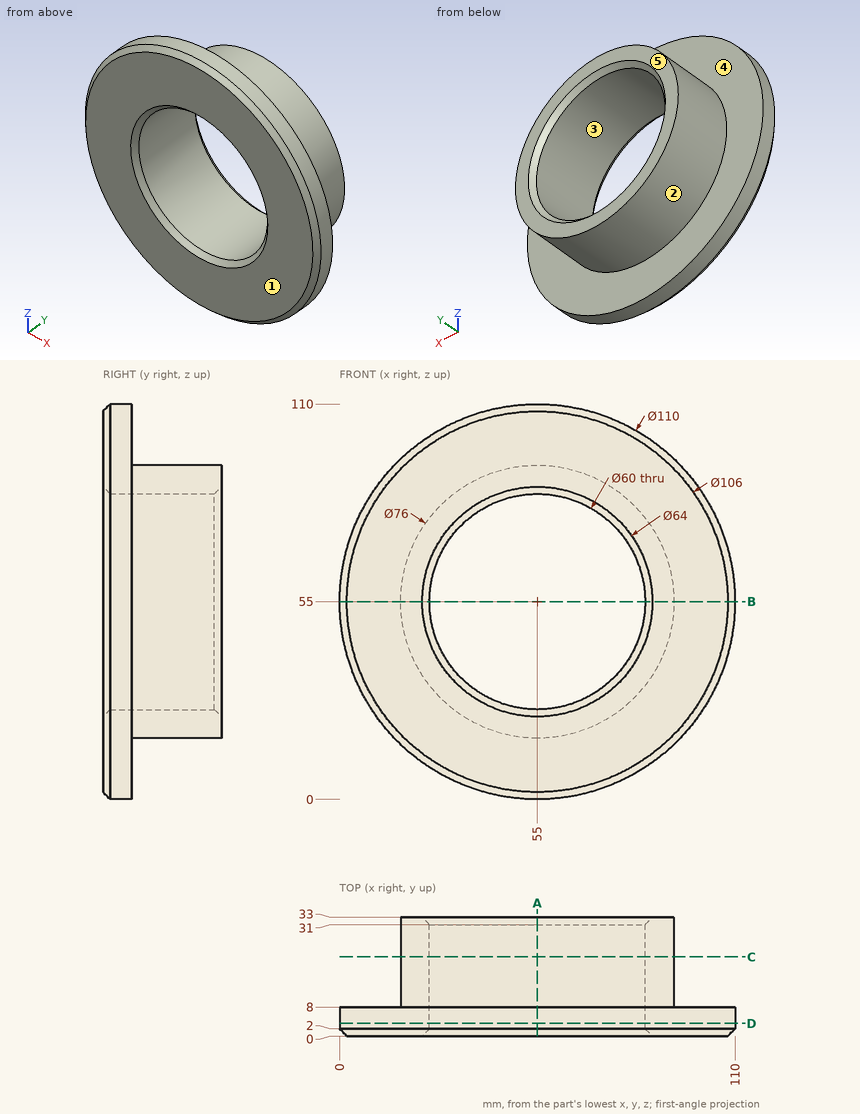
Input: dimensioned drawing with shaded views. Units: mm. Origin: part minimum x, y, z. A direction names the side the tool comes from. Coordinates: 2 decimals unless noted, no trailing zeros. Loops run counter-clockwise (first coordinate to the right, second up) from the corner with the lowest first, then second, coordinate; pieces in that order, holes last. Notation, with made-up numbers: (77.5, -38) -> (118.5, -38) arc R14 cw to (118.5, -13) -> close; hole circle Ø7 at (40, -28.75). An arc over 180 degrees is marked (long way). Use a Markdown table: item, result. Add a question column.
(1) Section query D-D, the plane y = 3.5. Return loops of the section in (x, z).
(2) Section query B-B, the plane z = 55. Return loops of the section in (x, y).
(3) Section query C-C, the plane y = 22. Return loops of the section in (x, z).
(4) Pin query (flat end, axial travel): pin 1 Ø2 at (x, z) = (13.5, 50) entering from -Y; pin 2 Ø4 at (x, y) = (36, 18.5) entering from -Z; pin 3 Ø1 at (y, z) = (24.5, 80) entering from +X; pin 4 Ø12 at (x, y) = (48.5, 22) entering from +Z. Return the tip coordinate at first contact, or that it passes through.
(5) Mould query, pull axis Z, two halves, no side actions, for the marked faces 1, 2 and 3. Classes: pulls with the +Z half, pulls with the -Z half, needs draft (parallel to the pull), parting line crosses it, or undercut.
(6) Line query: line 1 along X through (y, z) = (22, 55); line 2 along Y through (x, z) = (68.5, 98); line 3 along X through (y, z) = (20.5, 64.5). Output: solid intervals per line, ascending.
(7) Access query for the marked faces 4 and 5. Directions: +Z, -Z, +X, -X, +Y, -Y. A direction counts if a zero-diameter tool reaches every point of the face in a straight line with its end or side. Return the directions, or none.
(8) Section query A-A, the plane x = 55. Return loops of the section in (y, z).
Answer:
| question | item | result |
|---|---|---|
| 1 | outline | circle Ø110 at (55, 55); hole circle Ø60 at (55, 55) |
| 2 | outline | (0, 2) -> (2, 0) -> (23, 0) -> (25, 2) -> (25, 31) -> (23, 33) -> (17, 33) -> (17, 8) -> (0, 8) -> close; (85, 2) -> (87, 0) -> (108, 0) -> (110, 2) -> (110, 8) -> (93, 8) -> (93, 33) -> (87, 33) -> (85, 31) -> close |
| 3 | outline | circle Ø76 at (55, 55); hole circle Ø60 at (55, 55) |
| 4 | pin 1 | stops at y = 0 |
| 4 | pin 2 | stops at z = 21.01 |
| 4 | pin 3 | stops at x = 84.05 |
| 4 | pin 4 | stops at z = 93 |
| 5 | face 1 | needs draft |
| 5 | face 2 | parting line crosses it |
| 5 | face 3 | undercut |
| 6 | line 1 | x = 17 to 25, 85 to 93 |
| 6 | line 2 | y = 0 to 8 |
| 6 | line 3 | x = 18.21 to 26.54, 83.46 to 91.79 |
| 7 | face 4 | +Y |
| 7 | face 5 | +Z, -Z, +X, -X, +Y |
| 8 | outline | (0, 2) -> (2, 0) -> (8, 0) -> (8, 17) -> (33, 17) -> (33, 23) -> (31, 25) -> (2, 25) -> (0, 23) -> close; (0, 87) -> (2, 85) -> (31, 85) -> (33, 87) -> (33, 93) -> (8, 93) -> (8, 110) -> (2, 110) -> (0, 108) -> close |
